Input: part model. Units: mm. Frame: model coordinates. A direction names the side the tool comes from. Coordinates: 2 decimals unless noted, no trailing zeros. Order: outer loops, then holes, each group sorted by start corner. A loop starts at its lowest first (then second) coordinate and runs counter-clockwise, first axis right, second up. Notation, with made-up numbers: M -37.5,-18 L 20.5,-18 A20 cw 20.5,-2 Z; hole C 44.5,31 d6. An arc over 180 degrees is marked long. One line per item, written item: value.
```python
from build123d import *

# Parameters (mm, degrees)
SKETCH1_R           = 35
SKETCH1_R_2         = 15
BOSS_EXTRUDE1_DEPTH = 20
SKETCH2_R           = 20
SKETCH2_R_2         = 15
BOSS_EXTRUDE2_DEPTH = 5
BOSS_EXTRUDE3_START = 20
SKETCH5_R           = 35
BOSS_EXTRUDE3_DEPTH = 20
BOSS_EXTRUDE4_START = 10
SKETCH6_R           = 20
BOSS_EXTRUDE4_DEPTH = 10


with BuildPart() as part:
    # Sketch1 → Boss-Extrude1 (new body)
    with BuildSketch(Plane.XY):
        Circle(SKETCH1_R)
        Circle(SKETCH1_R_2, mode=Mode.SUBTRACT)
    extrude(amount=BOSS_EXTRUDE1_DEPTH)

    # Sketch2 → Boss-Extrude2 (add, symmetric)
    with BuildSketch(Plane(origin=(0, 0, 0), x_dir=(-1, 0, 0), z_dir=(0, 0, -1))):
        with Locations(Location((0, 0, 0), (0, 0, 180))):
            Circle(SKETCH2_R)
        Circle(SKETCH2_R_2, mode=Mode.SUBTRACT)
    extrude(amount=BOSS_EXTRUDE2_DEPTH, both=True)

    # Sketch5 → Boss-Extrude3 (add)
    with BuildSketch(Plane(origin=(0, 0, -5), x_dir=(-1, 0, 0), z_dir=(0, 0, -1)).offset(BOSS_EXTRUDE3_START)):
        with Locations(Location((0, 0, 0), (0, 0, 180))):
            Circle(SKETCH5_R)
    extrude(amount=-BOSS_EXTRUDE3_DEPTH)

    # Sketch6 → Boss-Extrude4 (add)
    with BuildSketch(Plane(origin=(0, 0, -25), x_dir=(-1, 0, 0), z_dir=(0, 0, -1)).offset(BOSS_EXTRUDE4_START)):
        with Locations(Location((0, 0, 0), (0, 0, 180))):
            Circle(SKETCH6_R)
    extrude(amount=-BOSS_EXTRUDE4_DEPTH)

    # Sketch11 → Cut-Revolve2 (revolve, cut)
    with BuildSketch(Plane.XY.offset(-15)):
        Polygon((-11.623419421, 13.852251853), (-23.246838841, 27.704503705), (-19.416616626, 30.918441754), (-7.793197205, 17.066189901), align=None)
    revolve(axis=Axis((-11.623419421, 13.852251853, -15), (-0.642787609686535, 0.7660444431189817, 0)), mode=Mode.SUBTRACT)

    # Sketch17 → Cut-Revolve3 (revolve, cut)
    with BuildSketch(Plane.XY.offset(-15)):
        Polygon((12.450815126, 14.838303658), (24.416664753, 29.098647939), (28.246886969, 25.88470989), (16.281037342, 11.624365609), align=None)
    revolve(axis=Axis((12.450815126, 14.838303658, -15), (0.6427876096865406, 0.766044443118977, 0)), mode=Mode.SUBTRACT)


solid = part.part
```
(1) Cut plane D-D on y = -19. Output: boundary loops of the cut face in (x, z) (3 decimals), plus the area to 3 significant figures.
Data:
outline: M -29.394,-25 L -6.245,-25 L -6.245,-35 L 6.245,-35 L 6.245,-25 L 29.394,-25 L 29.394,-5 L 6.245,-5 L 6.245,0 L 29.394,0 L 29.394,20 L -29.394,20 L -29.394,0 L -6.245,0 L -6.245,-5 L -29.394,-5 Z
area: 2,540 mm2
(2) Cut plane A-A on z = 4. Output: boundary loops of the cut face in (x, y), plus the area to 3 significant figures.
Data:
outline: C 0,0 d70; hole C 0,0 d30
area: 3,140 mm2
(3) Draft query along Z for faces 5 (the flat face through (15, 15, -25)), 6 (the flat face through (15, -7, 20)), 7 (the flat face through (-11.677, 13.807, -15.07)), 8 (the cylindrical face through (-17.82, 19.54, -10.12)). Return one class per face: released by +Z, released by -Z, zero draft, split by the parting line, or undercut.
Data:
face 5: released by -Z
face 6: released by +Z
face 7: undercut
face 8: undercut
(4) Access query for faces 1 (the cylindrical face through (-19.98, -0.88, -2.54)), 2 (the flat face through (0, 0, -5)), 3 (the cylindrical face through (-19.98, -0.88, -30.07)), 4 (the cylindrical face through (-28, -21, 10)). Directions: +Z, -Z, +X, -X, +Y, -Y. A direction counts if a zero-diameter tool reaches every point of the face in a straight line with its end or side. Return the directions, or none.
Data:
face 1: none
face 2: +Z
face 3: -Z
face 4: +Z, -Z
(5) Ray query, line 1 (Z direction, x = 19, y = -25.5); line 2 (Y direction, x = 0, z = 10.5); line 3 (Y direction, x = 0, z = -2.3). Return the intervals inside material, ascending. Write a range as from..to.
Data:
line 1: z = -25..-5, 0..20
line 2: y = -35..-15, 15..35
line 3: y = -20..-15, 15..20
(6) Cut plane B-B on x = 0. Output: boundary loops of the cut face in (y, z).
Data:
outline: M -35,-25 L -20,-25 L -20,-35 L 20,-35 L 20,-25 L 35,-25 L 35,-5 L 20,-5 L 20,0 L 35,0 L 35,20 L 15,20 L 15,-5 L -15,-5 L -15,20 L -35,20 L -35,0 L -20,0 L -20,-5 L -35,-5 Z
(7) Cut plane C-C on z = -19. Output: boundary loops of the cut face in (x, y).
Data:
outline: M -24.71,24.78 A35 ccw long 24.71,24.78 L 14.75,12.91 L 10.15,16.77 L 20.12,28.64 A35 ccw -20.12,28.64 L -9.33,15.78 L -13.92,11.92 Z
(8) First-contact query: pin 1 (15 mm diameter, centred on x = -7, y = 1.5, fed in from +Z); pin 2 (3 mm diameter, centred on x = -23, z = 7, fed in from -Y); pin 3 (5 mm diameter, centred on x = -13.5, z = -28.5, fed in from -Y). Flat tips, straight axial feed; report the tip coordinate or a pass-through.
Data:
pin 1: stops at z = -5
pin 2: stops at y = -27.62
pin 3: stops at y = -16.7
